```python
from build123d import *

# Parameters (mm, degrees)
HEX_BODY_155AF_X65_DEPTH = 65
COLLAR_PROFILE_100_R     = 50
COLLAR_100_X50_DEPTH     = 50
THROUGH_BORE_75_REACH    = 167.044
BORE_PROFILE_75_R        = 37.5


with BuildPart() as part:
    # Hex Profile 155AF → Hex Body 155AF x65 (new body)
    with BuildSketch(Plane(origin=(0, 0, 0), x_dir=(1, 0, 0), z_dir=(0, 1, 0))):
        Polygon((89.489291724, 0), (44.744645862, 77.5), (-44.744645862, 77.5), (-89.489291724, 0), (-44.744645862, -77.5), (44.744645862, -77.5), align=None)
    extrude(amount=HEX_BODY_155AF_X65_DEPTH)

    # Hex Chamfer Profile 10x10 → Hex Corner Chamfer 10x10 (revolve, cut)
    with BuildSketch(Plane.XY):
        Polygon((79.489291724, 65), (89.489291724, 65), (89.489291724, 55), align=None)
    revolve(axis=Axis((0, 0, 0), (0, 1, 0)), mode=Mode.SUBTRACT)

    # Collar Profile Ø100 → Collar Ø100 x50 (add)
    with BuildSketch(Plane(origin=(0, 65, 0), x_dir=(1, 0, 0), z_dir=(0, 1, 0))):
        with Locations(Location((0, 0, 0), (0, 0, 270))):
            Circle(COLLAR_PROFILE_100_R)
    extrude(amount=COLLAR_100_X50_DEPTH)

    # Bore Profile Ø75 → Through Bore Ø75 (cut, up to next)
    with BuildSketch(Plane(origin=(0, 115, 0), x_dir=(1, 0, 0), z_dir=(0, 1, 0)), mode=Mode.PRIVATE) as through_bore_75_sk1:
        with Locations(Location((0, 0, 0), (0, 0, 270))):
            Circle(BORE_PROFILE_75_R)
    through_bore_75_tool1 = extrude(through_bore_75_sk1.sketch, amount=-THROUGH_BORE_75_REACH, mode=Mode.PRIVATE) & part.part
    add(through_bore_75_tool1.solids().sort_by_distance((0, 115, 0))[0], mode=Mode.SUBTRACT)


solid = part.part
```
CAD build for the part. Positions are in the model's coordinates, mm. A direction names the side the tool comes from. Round coordinates to 2 decimals unless told otherwise and drop trailing zeros. Order: outer loops, then holes, each group sorted by start corner. A loop starts at its lowest first (then second) coordinate and runs counter-clockwise, first axis right, second up. Notation, with made-up numbers: (86.25, 70.5) - (109.25, 70.5) arc R28 cw to (109.25, 90.5) - close; hole circle Ø1 at (-6, 12). An arc over 180 degrees is marked (long way). Answer in a Markdown table with one row per item. Add a question column.
(1) Band-saw the part on C-C on z = -40. List the corners of the cut face in (x, y).
(2) Band-saw the part on A-A on x = 0. List the corners of the cut face in (y, z).
(3) Band-saw the part on D-D on y = 57.5. List the corners of the cut face in (x, z), and give its area (3 significant figures).
(4) Band-saw the part on B-B on y = 23.5. List the corners of the cut face in (x, z), and give its area (3 significant figures).
(5) 3-axis set-ups, long thin cutter, end or side, ignore diameter. For faces 1 (the face through (-66.8, 32, -39.3)), 2 (the face through (15.02, 89.65, 47.69)): which of +Z, -Z, +X, -X, +Y, -Y reach the whole face in a straight line?
(6) Mould opens along Z. For faces 3 (the face through (-41.4, 62.3, 71)), 4 (the face through (-22.818, 58.305, -29.759)), 5 (the face through (82.2, 62.29, 0.34)), 6 (the face through (1, 32, -77.5)) say: +Z half, -Z half, draft (parallel to the pull), parting line (faces both ways), or undercut.
(7) Drop flat-ended pins along their axis: pin 1 Ø10 at (y, z) = (90.5, 44) entering from -X; pin 2 Ø2 at (y, z) = (33.5, 6.5) entering from +X; pin 3 Ø3 at (y, z) = (72.5, 25) entering from -X. Give the stop position or say it passes through.
(8) Probe L1, parallel to X at y = 69, z = 0; L2, parallel to X at y = 42.5, z = 0. List the from-to ranges inside material, lowest first. Write a range as [from, to].
Data:
| question | item | result |
|---|---|---|
| 1 | outline | (-66.4, 0) - (66.4, 0) - (66.4, 65) - (30, 65) - (30, 115) - (-30, 115) - (-30, 65) - (-66.4, 65) - close |
| 2 | outline | (0, -77.5) - (65, -77.5) - (65, -50) - (115, -50) - (115, -37.5) - (0, -37.5) - close; (0, 37.5) - (115, 37.5) - (115, 50) - (65, 50) - (65, 77.5) - (0, 77.5) - close |
| 3 | outline | (-86.87, -4.54) - (-47.36, -72.96) arc R86.99 ccw to (-39.51, -77.5) - (39.51, -77.5) arc R86.99 ccw to (47.36, -72.96) - (86.87, -4.54) arc R86.99 ccw to (86.87, 4.54) - (47.36, 72.96) arc R86.99 ccw to (39.51, 77.5) - (-39.51, 77.5) arc R86.99 ccw to (-47.36, 72.96) - (-86.87, 4.54) arc R86.99 ccw to start; hole circle Ø75 at (0, 0) |
| 3 | area | 16,300 mm^2 |
| 4 | outline | (-89.49, 0) - (-44.74, -77.5) - (44.74, -77.5) - (89.49, 0) - (44.74, 77.5) - (-44.74, 77.5) - close; hole circle Ø75 at (0, 0) |
| 4 | area | 16,400 mm^2 |
| 5 | face 1 | -Z, -X, +Y, -Y |
| 5 | face 2 | +Y |
| 6 | face 3 | +Z half |
| 6 | face 4 | undercut |
| 6 | face 5 | parting line |
| 6 | face 6 | -Z half |
| 7 | pin 1 | stops at x = -31.29 |
| 7 | pin 2 | stops at x = 86.31 |
| 7 | pin 3 | stops at x = -44.13 |
| 8 | L1 | x = [-50, -37.5], [37.5, 50] |
| 8 | L2 | x = [-89.49, -37.5], [37.5, 89.49] |
